Geometry check sheet. Reference: the model listing, model coordinates, mm. A direction names the side the tool comes from. Round coordinates to 2 decimals unless told otherwise and drop trailing zeros. Write each loop counter-clockwise with the first axis right and the second up, starting at its lowest first coordinate (ties: lowest second). Pieces come first, ordered by that corner, then holes. Notation, with made-up numbers: M -12.75,24 L -5.75,24 A4 ccw -5.75,29 Z; hole C 42,-8 d3. An arc over 180 degrees is marked long. One line per item, written item: value. Start each with the question number.
1. Section check D-D (y = 31). Record the boundary of the cut face in (x, z), and give its area (3 significant figures).
2. Scan lines: probe 1 along X at (y, z) = (46.5, -12.5); probe 2 along Z at (x, y) = (13, 51.5); probe 3 along X at (y, z) = (40, -10). Record each from-to range of solid material in increasing order. Write a range as [from, to].
3. Section check A-A (z = 3.5). Record the boundary of the cut face in (x, y).
4. Depth check by flat-ended pin: P1, Ø4, axis at x = 5, z = 9, coming from the -Y side; P2, Ø2, axis at x = 11.5, z = -5.5, coming from the +Y side; P3, Ø3, axis at x = 0.5, z = -4.5, coming from the +Y side. Enter the tip coordinate at first touch or a pass-through.
5. Release check for a two-part mould opening along Y. For faces 1 (the cylindrical face through (-8.41, 46.82, 12.82)), 2 (the conical face through (-9.56, 33.996, -13.399)), 3 (the flat face through (-15.3, 26.5, 0.4)), 4 (the flat face through (2.75, 20, 0)) record: pulls with the +Y half, pulls with the -Y half, needs draft (parallel to the pull), parting line crosses it, or undercut.
6. Access from +Z, -Z, +X, -X, +Y, -Y to the whole of each face (thin tool, end or side, straight path). Record for faces 5 (the flat face through (0, 36, 20.3)), 6 (the flat face through (-2.75, 20, 0)), 7 (the flat face through (0, 36, -20.3)), 8 (the flat face through (15.3, 26.5, 0.4)), 9 (the cylindrical face through (5.805, 16.509, 0.35)).
7. Section check C-C (y = 39). Count the separate pieces of the cut face and the enclosed holes in it, and give its area (3 significant figures).
8. Section check B-B (x = -2). Record the boundary of the cut face in (y, z), and give its area (3 significant figures).
from build123d import *

# Parameters (mm, degrees)
BOSS_EXTRUDE1_DEPTH                       = 25
BOSS_EXTRUDE1_2_DEPTH                     = 25
SKETCH2_W                                 = 5.5
SKETCH2_H                                 = 28.1
BOSS_EXTRUDE2_DEPTH                       = 20.3
F_8_0MM_BLIND_DOWEL_HOLE1_D               = 8
F_8_0MM_BLIND_DOWEL_HOLE1_DEPTH           = 15
F_8_0MM_BLIND_DOWEL_HOLE1_TIP             = 2.403442476
F_8_0MM_BLIND_DOWEL_HOLE1_ON_FACE_2_D     = 8
F_8_0MM_BLIND_DOWEL_HOLE1_ON_FACE_2_DEPTH = 15
F_8_0MM_BLIND_DOWEL_HOLE1_ON_FACE_2_TIP   = 2.403442476
M8_TAPPED_HOLE1_D                         = 6.8
M8_TAPPED_HOLE1_DEPTH                     = 18
M8_TAPPED_HOLE1_TIP                       = 2.042926105
M8_TAPPED_HOLE1_ON_FACE_2_D               = 6.8
M8_TAPPED_HOLE1_ON_FACE_2_DEPTH           = 18
M8_TAPPED_HOLE1_ON_FACE_2_TIP             = 2.042926105


with BuildPart() as part:
    # Sketch1 → Boss-Extrude1 (new, symmetric)
    with BuildSketch(Plane.XY):
        with BuildLine():
            Line((-8.75, 15.155444566), (-22, 38.105117767))
            Line((-22, 38.105117767), (-22, 50.408332645))
            ThreePointArc((-22, 50.408332645), (-12.579933349, 53.541995452), (-2.75, 54.931206977))
            Line((-2.75, 54.931206977), (-2.75, 17.282577933))
            ThreePointArc((-2.75, 17.282577933), (-5.847535728, 16.494130044), (-8.75, 15.155444566))
        make_face()
    extrude(amount=BOSS_EXTRUDE1_DEPTH, both=True)



with BuildPart() as body_2:
    # Sketch1 → Boss-Extrude1 2 (new, symmetric)
    with BuildSketch(Plane.XY):
        with BuildLine():
            Line((8.75, 15.155444566), (22, 38.105117767))
            Line((22, 38.105117767), (22, 50.408332645))
            ThreePointArc((22, 50.408332645), (12.579933349, 53.541995452), (2.75, 54.931206977))
            Line((2.75, 54.931206977), (2.75, 17.282577933))
            ThreePointArc((2.75, 17.282577933), (5.847535728, 16.494130044), (8.75, 15.155444566))
        make_face()
    extrude(amount=BOSS_EXTRUDE1_2_DEPTH, both=True)


with BuildPart() as part_1:
    add(part.part)

    add(body_2.part)  # Boss-Extrude2 merges body 2
    # Sketch2 → Boss-Extrude2 (add, symmetric)
    with BuildSketch(Plane.XY):
        with Locations((0, 36.25)):
            Rectangle(SKETCH2_W, SKETCH2_H)
    extrude(amount=BOSS_EXTRUDE2_DEPTH, both=True)

    # Ø8.0mm Blind Dowel Hole1
    with Locations(Plane(origin=(-14.235047481, 53.125920446, 13), x_dir=(0.965925826289, 0.258819045103, 0), z_dir=(-0.258819045103, 0.965925826289, 0))):
        with Locations((0, 0)):
            Hole(F_8_0MM_BLIND_DOWEL_HOLE1_D / 2, depth=F_8_0MM_BLIND_DOWEL_HOLE1_DEPTH)
            with Locations((0, 0, -(F_8_0MM_BLIND_DOWEL_HOLE1_DEPTH + F_8_0MM_BLIND_DOWEL_HOLE1_TIP / 2))):  # 118° drill point
                Cone(0, F_8_0MM_BLIND_DOWEL_HOLE1_D / 2, F_8_0MM_BLIND_DOWEL_HOLE1_TIP, mode=Mode.SUBTRACT)

    # Ø8.0mm Blind Dowel Hole1 on face 2
    with Locations(Plane(origin=(14.235047481, 53.125920446, -13), x_dir=(0.965925849201, -0.258818959594, 0), z_dir=(0.258818959594, 0.965925849201, 0))):
        with Locations((0, 0)):
            Hole(F_8_0MM_BLIND_DOWEL_HOLE1_ON_FACE_2_D / 2, depth=F_8_0MM_BLIND_DOWEL_HOLE1_ON_FACE_2_DEPTH)
            with Locations((0, 0, -(F_8_0MM_BLIND_DOWEL_HOLE1_ON_FACE_2_DEPTH + F_8_0MM_BLIND_DOWEL_HOLE1_ON_FACE_2_TIP / 2))):  # 118° drill point
                Cone(0, F_8_0MM_BLIND_DOWEL_HOLE1_ON_FACE_2_D / 2, F_8_0MM_BLIND_DOWEL_HOLE1_ON_FACE_2_TIP, mode=Mode.SUBTRACT)

    # M8 Tapped Hole1
    with Locations(Plane(origin=(-14.235047481, 53.125920446, -13), x_dir=(0.965925826289, 0.258819045103, 0), z_dir=(-0.258819045103, 0.965925826289, 0))):
        with Locations((0, 0)):
            Hole(M8_TAPPED_HOLE1_D / 2, depth=M8_TAPPED_HOLE1_DEPTH)
            with Locations((0, 0, -(M8_TAPPED_HOLE1_DEPTH + M8_TAPPED_HOLE1_TIP / 2))):  # 118° drill point
                Cone(0, M8_TAPPED_HOLE1_D / 2, M8_TAPPED_HOLE1_TIP, mode=Mode.SUBTRACT)

    # M8 Tapped Hole1 on face 2
    with Locations(Plane(origin=(14.235047481, 53.125920446, 13), x_dir=(0.965925849201, -0.258818959594, 0), z_dir=(0.258818959594, 0.965925849201, 0))):
        with Locations((0, 0)):
            Hole(M8_TAPPED_HOLE1_ON_FACE_2_D / 2, depth=M8_TAPPED_HOLE1_ON_FACE_2_DEPTH)
            with Locations((0, 0, -(M8_TAPPED_HOLE1_ON_FACE_2_DEPTH + M8_TAPPED_HOLE1_ON_FACE_2_TIP / 2))):  # 118° drill point
                Cone(0, M8_TAPPED_HOLE1_ON_FACE_2_D / 2, M8_TAPPED_HOLE1_ON_FACE_2_TIP, mode=Mode.SUBTRACT)


solid = part_1.part
Result sheet:
1. outline: M -17.9,-25 L -2.75,-25 L -2.75,-20.3 L 2.75,-20.3 L 2.75,-25 L 17.9,-25 L 17.9,25 L 2.75,25 L 2.75,20.3 L -2.75,20.3 L -2.75,25 L -17.9,25 Z
1. area: 1,740 mm2
2. probe 1: x = [-22, -15.94], [-8.98, 8.35], [16.57, 22]
2. probe 2: z = [-25, -16.92], [-9.08, 9.69], [16.31, 25]
2. probe 3: x = [-22, -12.37], [-9.06, 7.98], [13.46, 22]
3. outline: M -22,38.11 L -8.75,15.16 A17.5 cw -2.75,17.28 L -2.75,22.2 L 2.75,22.2 L 2.75,17.28 A17.5 cw 8.75,15.16 L 22,38.11 L 22,50.41 A55 ccw 2.75,54.93 L 2.75,50.3 L -2.75,50.3 L -2.75,54.93 A55 ccw -22,50.41 Z
4. P1: stops at y = 16.04
4. P2: stops at y = 53.99
4. P3: stops at y = 50.3
5. face 1: undercut
5. face 2: undercut
5. face 3: pulls with the -Y half
5. face 4: needs draft
6. face 5: +Z, +Y, -Y
6. face 6: none
6. face 7: -Z, +Y, -Y
6. face 8: +Z, -Z, +X, -Y
6. face 9: +Z, -Z, -Y
7. separate pieces: 1
7. enclosed holes: 4
7. area: 1,980 mm2
8. outline: M 22.2,-20.3 L 50.3,-20.3 L 50.3,20.3 L 22.2,20.3 Z
8. area: 1,140 mm2
